For this review, take the finished solid that the model builds, in its own axes (mm). A direction names the side the tool comes from. Give positions to 0.01 mm unless a question says otherwise; leave off trailing zeros. Write each loop counter-clockwise with the first axis right and the second up, starting at its lowest first coordinate (ties: lowest second). Pieces come first, ordered by that corner, then holes. Notation, with made-up numbers: M -21,-16.75 L -10,-16.75 A18 cw -10,2.25 Z; hole C 83.25,-3.75 d8. An arc over 180 degrees is marked long. One line per item, written item: value. Start each with the question number.
Item 1: To check wall thickness, follow probe 1 along Y at (x, z) = (-0.2, -210); probe 2 along Z at (x, y) = (0.35, -21); probe 3 along Z at (x, y) = (-1.5, -10.5). State the ranges of each line that lie inside material, in increasing order.
Item 2: Consider section A-A, the plane x = 0.5. Write out the cut boundary in (y, z), and give its area (3 significant figures).
Item 3: Tool access review of faces 1 (the face through (-3.913, -56.986, -99.852)), 2 (the face through (3.866, 15.053, -101.495)), 3 (the face through (-0.039, 12.285, -102.461)): name each direction out of +Z, -Z, +X, -X, +Y, -Y from which nothing blocks a thin tool from reaching the whole face with its end or side.
Item 4: Clearance check with flat-ended pins moving along their axes: pin 1 Ø1 at (x, y) = (-3.5, -4.5) entering from -Z; pin 2 Ø1 at (x, z) = (-2, -160.5) entering from -Y; pin 3 Ø3 at (x, z) = (2.5, -6) entering from +Y. State where each tip first meets the part, or that it passes through.
Item 5: Mouldability with a two-part tool opening along Z and no side actions: class faces 4 (the face through (3.866, -56.86, -99.883)), 5 (the face through (-0.07, -20.848, 26.817)) as released by +Z, released by -Z, zero draft, split by the parting line, or undercut.
Item 6: Consider section B-B, the plane z = -80.5. Write out the cut boundary in (x, y).
```python
from build123d import *


with BuildPart() as part:
    # Sweep1: sweep along a path in Sketch3
    with BuildLine(Plane(origin=(0, 0, 0), x_dir=(0, 0, -1), z_dir=(1, 0, 0))) as sweep1_path:
        Line((-2.5, -0.149340538), (204.523809524, 24.672873107))
        ThreePointArc((204.523809524, 24.672873107), (256, -21), (204.523809524, -66.672873107))
        Line((204.523809524, -66.672873107), (-2.5, -41.850659462))
        ThreePointArc((-2.5, -41.850659462), (-21, -21), (-2.5, -0.149340538))
    # Sketch2 → Sweep1 (sweep)
    with BuildSketch(Plane.XY):
        Polygon((-5, 6), (5, 6), (2.816178594, 0), (-2.816178594, 0), align=None)
    sweep(path=sweep1_path.line)


solid = part.part
```
Model answer:
1. probe 1: y = -72.81 to -66.85, 24.85 to 30.81
1. probe 2: z = -261.81 to -255.85, 20.85 to 26.82
1. probe 3: z = -260.74 to -254.63, 18.01 to 24.68
2. outline: M -72.36,-203.14 A51.81 ccw long 30.52,-204.52 L 5.7,2.5 A26.82 ccw -47.53,3.88 Z; hole M -66.53,-204.56 A45.85 ccw long 24.52,-204.52 L -0.3,2.5 A20.85 ccw -41.7,2.46 Z
2. area: 3,880 mm2
3. face 1: -X
3. face 2: +X
3. face 3: +X, -X
4. pin 1: stops at z = -259.28
4. pin 2: stops at y = -67.3
4. pin 3: stops at y = 6.9
5. face 4: undercut
5. face 5: released by +Z
6. outline: M -5,-57.65 L 5,-57.65 L 2.82,-51.65 L -2.82,-51.65 Z; M -5,15.65 L -2.82,9.65 L 2.82,9.65 L 5,15.65 Z
